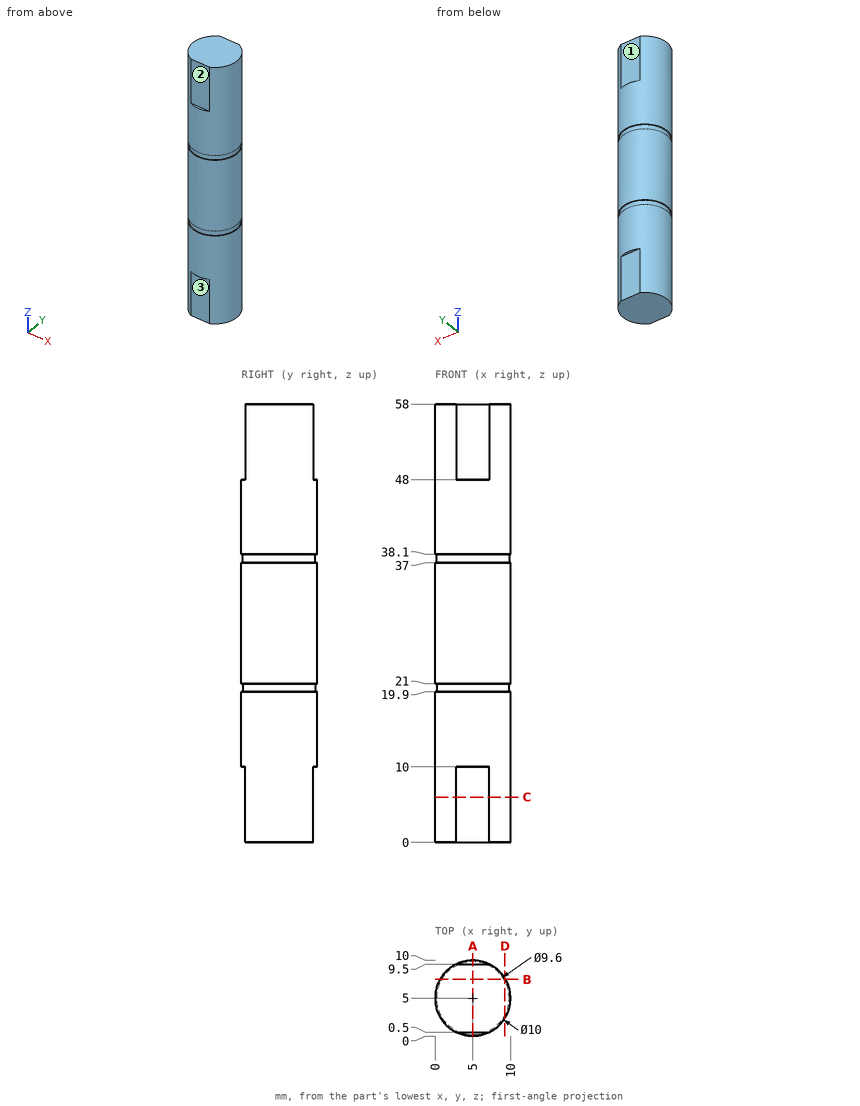
Print and shaded views of the part. All mm, measured from the part's lowest x, y and z. A direction names the side the tool comes from. Coordinates: 2 decimals unless noted, no trailing zeros. Order: outer loops, then holes, each group sorted by start corner. A loop starts at its lowest first (then second) coordinate and runs counter-clockwise, first axis right, second up.
Item 1: Drop flat-ended pins along their axis: pin 1 Ø1.3 at (x, z) = (5, 51) entering from +Y; pin 2 Ø0.6 at (x, y) = (4.5, 10) entering from -Z; pin 3 Ø2 at (x, z) = (3.5, 40.5) entering from +Y; pin 4 Ø6 at (x, y) = (5, 2.5) entering from -Z. Give the stop position or say it passes through.
Filled in:
pin 1: stops at y = 9.5
pin 2: stops at z = 10
pin 3: stops at y = 9.97
pin 4: stops at z = 0
Item 2: Saw through at D-D on x = 9.25. List the corners of the cut face in (y, z), then the cut area to 3 significant figures.
Filled in:
outline: (2.37, 0) - (7.63, 0) - (7.63, 19.9) - (7.23, 19.9) - (7.23, 21) - (7.63, 21) - (7.63, 37) - (7.23, 37) - (7.23, 38.1) - (7.63, 38.1) - (7.63, 58) - (2.37, 58) - (2.37, 38.1) - (2.77, 38.1) - (2.77, 37) - (2.37, 37) - (2.37, 21) - (2.77, 21) - (2.77, 19.9) - (2.37, 19.9) - close
area: 304 mm2
Item 3: Saw through at A-A on x = 5. List the corners of the cut face in (y, z), then the cut area to 3 significant figures.
Filled in:
outline: (0, 10) - (0.5, 10) - (0.5, 0) - (9.5, 0) - (9.5, 10) - (10, 10) - (10, 19.9) - (9.8, 19.9) - (9.8, 21) - (10, 21) - (10, 37) - (9.8, 37) - (9.8, 38.1) - (10, 38.1) - (10, 48) - (9.5, 48) - (9.5, 58) - (0.5, 58) - (0.5, 48) - (0, 48) - (0, 38.1) - (0.2, 38.1) - (0.2, 37) - (0, 37) - (0, 21) - (0.2, 21) - (0.2, 19.9) - (0, 19.9) - close
area: 559 mm2
Item 4: Saw through at C-C on z = 6. List the corners of the cut face in (x, y).
Filled in:
outline: (2.82, 0.5) - (7.18, 0.5) arc R5 ccw to (7.18, 9.5) - (2.82, 9.5) arc R5 ccw to start
Item 5: Saw through at B-B on y = 7.5. List the corners of the cut face in (x, z).
Filled in:
outline: (0.67, 0) - (9.33, 0) - (9.33, 19.9) - (9.1, 19.9) - (9.1, 21) - (9.33, 21) - (9.33, 37) - (9.1, 37) - (9.1, 38.1) - (9.33, 38.1) - (9.33, 58) - (0.67, 58) - (0.67, 38.1) - (0.9, 38.1) - (0.9, 37) - (0.67, 37) - (0.67, 21) - (0.9, 21) - (0.9, 19.9) - (0.67, 19.9) - close
Item 6: Tool access for the marked faces 1, 2 and 3: list every direction of +Z, -Z, +X, -X, +Y, -Y with a clear straight run to the whole face (end or side of a thin tool).
Filled in:
face 1: +Z, +X, -X, +Y
face 2: +Z, +X, -X, -Y
face 3: -Z, +X, -X, -Y
Item 7: Drill centre lines: L1, parallel to Z at x = 7.75, y = 1; L2, parallel to X at y = 5.25, z = 8.5; L3, parallel to Y at x = 9.5, z = 26.5. Where is each one in solid material? Low to high.
Filled in:
L1: z = 0 to 19.9, 21 to 37, 38.1 to 58
L2: x = 0.01 to 9.99
L3: y = 2.82 to 7.18
